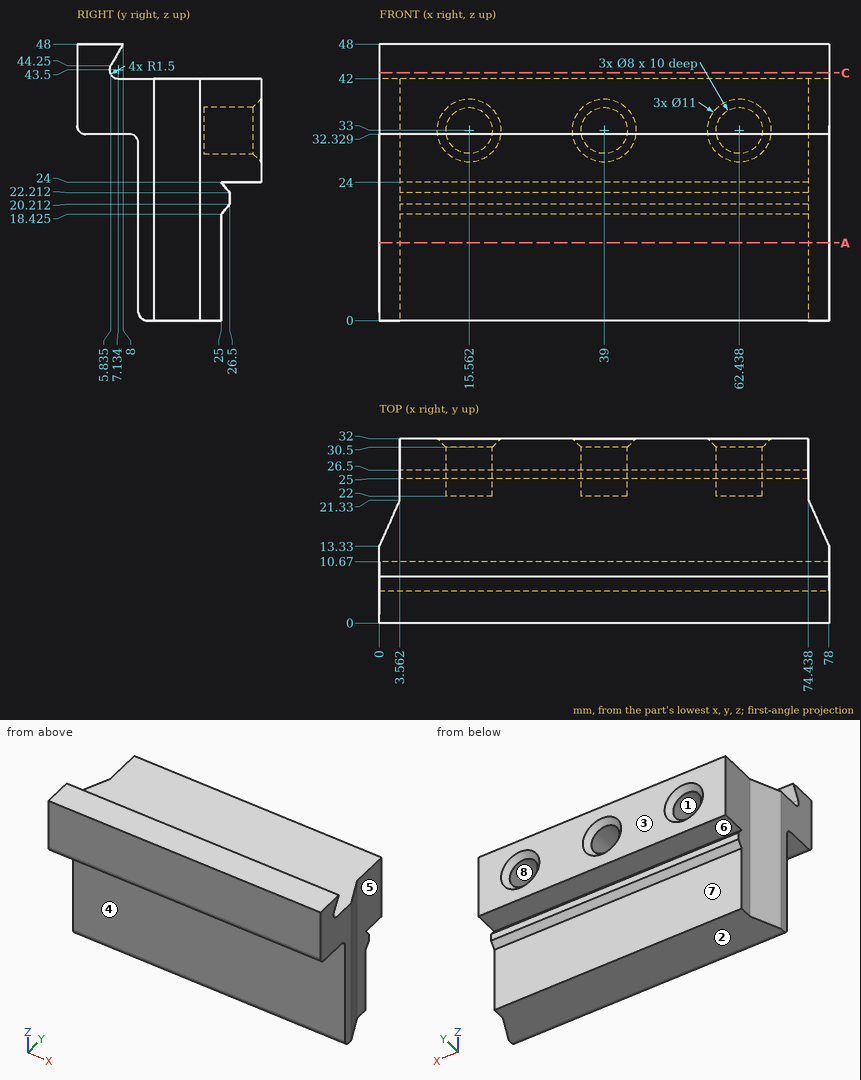
For this review, use the dimensioned drawing (mm, ordinates from the lowest corner) and the shaded views. A direction names the side the tool comes from. Give positions to 0.01 mm unless a question says otherwise; leave off trailing zeros. Order: outer loops, then holes, each group sorted by start corner. A loop starts at its lowest first (then second) coordinate and runs counter-clockwise, first axis right, second up.
1) For the marked faces 4, 5, 6, 7 and 8, list the 3-axis set-ups (+Z, -Z, +X, -X, +Y, -Y) from which the entire face can be reached by the end or side of a thin tool; tool diameter is ignored.
2) Take a section at A-A (z = 13.5). Give the boundary of the cut face in (x, y), then the cut area to 3 significant figures.
3) Wall thickness on line 1 (X direction, y = 25.25, z = 33); line 2 (Y direction, x = 30, z = 3); line 3 (Y direction, x = 58.5, z = 21): over which ranges is each line inside the solid? List them lowest first.
4) Insertion check: pin 1 (5.5 mm diameter, centred on x = 47.5, y = 27, fed in from -Z); pin 2 (1 mm diameter, centred on x = 13, z = 18.5, fed in from +Y); pin 3 (12 mm diameter, centred on x = 16, y = 20.5, fed in from +Z); pin 4 (8.5 mm diameter, centred on y = 27, z = 21.5, fed in from -X). Each pin has a flat end and moves straight along its axis. Give the tip position at first contact, or say it passes through.
5) The part is to be moulded in two halves that separate along Z. For the marked faces 1, 2 and 3, say which applies: released by +Z, released by -Z, zero draft, split by the parting line, or undercut.
6) Take a section at C-C (z = 43). Give the boundary of the cut face in (x, y), then the cut area to 3 significant figures.
Derived:
1. face 4: -Z, +X, -X, -Y
1. face 5: +Z, -Z, +X, +Y
1. face 6: +X, -X, +Y
1. face 7: -Z, +X, -X, +Y
1. face 8: +Y
2. outline: (0, 10.67) - (78, 10.67) - (78, 13.33) - (74.44, 21.33) - (74.44, 25) - (3.56, 25) - (3.56, 21.33) - (0, 13.33) - close
2. area: 1,060 mm2
3. line 1: x = 3.56 to 11.56, 19.56 to 35, 43 to 58.44, 66.44 to 74.44
3. line 2: y = 10.67 to 25
3. line 3: y = 10.67 to 26.5
4. pin 1: stops at z = 0
4. pin 2: stops at y = 25.48
4. pin 3: stops at z = 42
4. pin 4: stops at x = 3.56
5. face 1: undercut
5. face 2: released by -Z
5. face 3: zero draft
6. outline: (0, 0) - (78, 0) - (78, 5.72) - (0, 5.72) - close
6. area: 446 mm2
